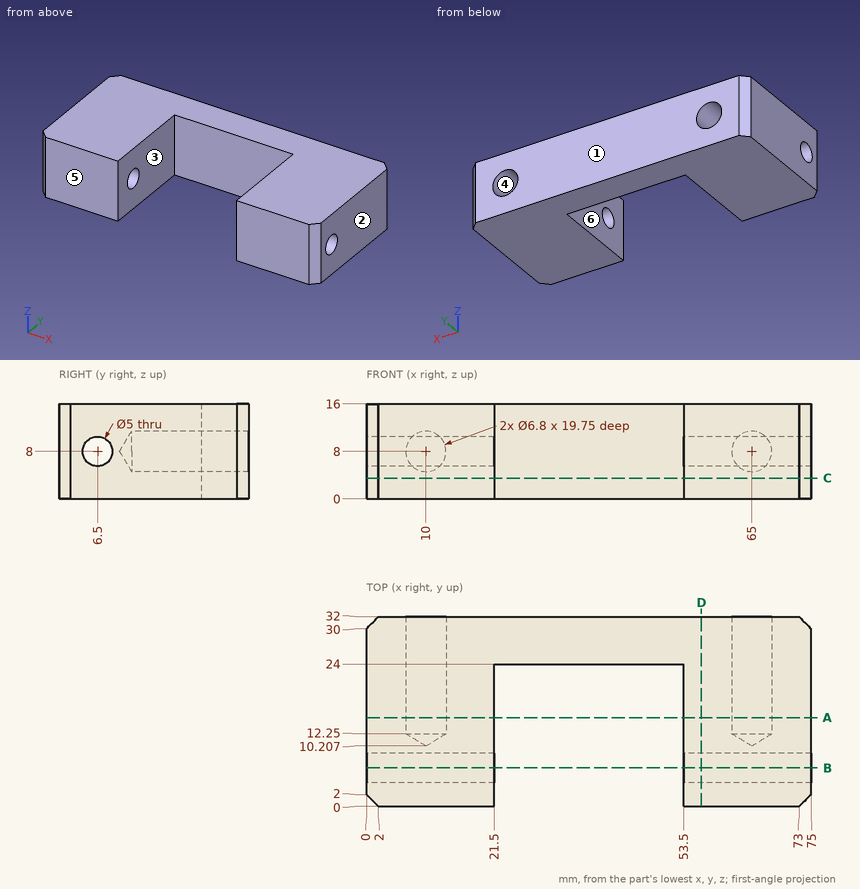
Drawing for the job (mm, zero at the part's lowest x, y, z). A direction names the side the tool comes from. Round coordinates to 2 decimals unless told otherwise and drop trailing zeros. Order: outer loops, then holes, each group sorted by start corner. A loop starts at its lowest first (then second) coordinate and runs counter-clockwise, first axis right, second up. Notation, with made-up numbers: M -25.75,17.25 L -21.75,17.25 A18 cw -21.75,27.25 Z; hole C 28.5,-2.75 d11. An arc over 180 degrees is marked long. Use one line per item in the form item = value.
Q1. Saw through at B-B on y = 6.5. Give the cut face in (x, z), then the cut area to 3 significant figures.
Recorded:
outline = M 0,0 L 21.5,0 L 21.5,5.5 L 0,5.5 Z; M 0,10.5 L 21.5,10.5 L 21.5,16 L 0,16 Z; M 53.5,0 L 75,0 L 75,5.5 L 53.5,5.5 Z; M 53.5,10.5 L 75,10.5 L 75,16 L 53.5,16 Z
area = 473 mm^2
Q2. Two-plate mould, pull along X, no slides. Class the marked faces 1, 2 and 3: +X half, -X half, draft (parallel to the pull), parting line (faces both ways), or undercut.
Recorded:
face_1 = draft
face_2 = +X half
face_3 = undercut
Q3. Flat gauge pins, fed straight in: P1, Ø5, axis at x = 30, z = 9, coming from the -Y side; P2, Ø4.5, axis at y = 6.5, z = 8, coming from the +X side (3 decimals). Where does each tip first touch, or does it go through?
Recorded:
P1 = 24
P2 = through
Q4. Which spindle directions (+Z, -Z, +X, -X, +Y, -Y) get a long thin tool onto all of the face, cutting with end or side? Do the marked faces 4, 5 and 6. Say none if no direction does.
Recorded:
face_4 = +Y
face_5 = +Z, -Z, +X, -X, -Y
face_6 = +Z, -Z, -Y
Q5. Saw through at A-A on y = 15. Give the cut face in (x, z), then the cut area to 3 significant figures.
Recorded:
outline = M 0,0 L 21.5,0 L 21.5,16 L 0,16 Z; M 53.5,0 L 75,0 L 75,16 L 53.5,16 Z; hole C 10,8 d6.8; hole C 65,8 d6.8
area = 615 mm^2
Q6. Saw through at D-D on x = 56.5. Give the cut face in (y, z).
Recorded:
outline = M 0,0 L 32,0 L 32,16 L 0,16 Z; hole C 6.5,8 d5
Q7. Saw through at C-C on z = 3.5. Give the cut face in (x, y).
Recorded:
outline = M 0,2 L 2,0 L 21.5,0 L 21.5,24 L 53.5,24 L 53.5,0 L 73,0 L 75,2 L 75,30 L 73,32 L 2,32 L 0,30 Z
Q8. Probe L1, parallel to X at y = 19, z = 8; L2, parallel to X at y = 2, z = 12; L3, parallel to X at y = 27.5, z = 10.5. List the from-to ranges inside material, lowest first.
Recorded:
L1 = 0 to 6.6, 13.4 to 21.5, 53.5 to 61.6, 68.4 to 75
L2 = 0 to 21.5, 53.5 to 75
L3 = 0 to 7.7, 12.3 to 62.7, 67.3 to 75
